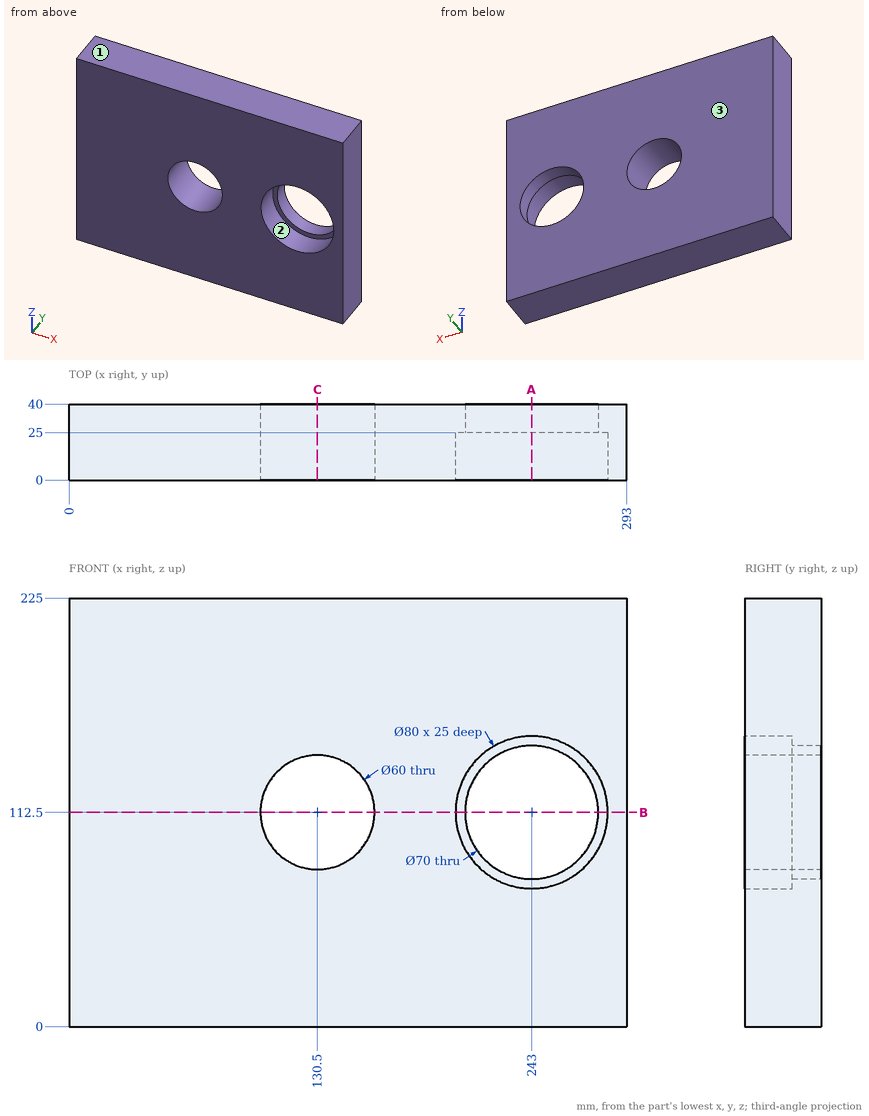
Input: dimensioned drawing with shaded views. Units: mm. Origin: part minimum x, y, z. Give positions to 0.01 mm unless a question says otherwise; leave off trailing zeros. Loops run counter-clockwise (first coordinate to the right, second up) from the corner with the lowest first, then second, coordinate; pieces in that order, holes last. Notation, with made-up numbers: (-7.75, -21) -> (22.25, -21) arc R21 cw to (22.25, 6) -> close; hole circle Ø11 at (-38.5, 42). An arc over 180 degrees is marked (long way). Use a Markdown table: item, result.
Q1. Section query A-A, the plane x = 243. Return the cut outline in (y, z).
Entries:
| item | result |
|---|---|
| outline | (0, 0) -> (40, 0) -> (40, 77.5) -> (25, 77.5) -> (25, 72.5) -> (0, 72.5) -> close; (0, 152.5) -> (25, 152.5) -> (25, 147.5) -> (40, 147.5) -> (40, 225) -> (0, 225) -> close |
Q2. Section query C-C, the plane x = 130.5. Return the cut outline in (y, z).
Entries:
| item | result |
|---|---|
| outline | (0, 0) -> (40, 0) -> (40, 82.5) -> (0, 82.5) -> close; (0, 142.5) -> (40, 142.5) -> (40, 225) -> (0, 225) -> close |
Q3. Pull-direction query (Z, two-part tool) for the marked faces 1, 2 and 3; classes: pulls with the +Z half, pulls with the -Z half, needs draft (parallel to the pull), parting line crosses it, or undercut.
Entries:
| item | result |
|---|---|
| face 1 | pulls with the +Z half |
| face 2 | undercut |
| face 3 | needs draft |
Q4. First-contact query: P1, Ø5, axis at y = 16, z = 58, coming from the -X side; P2, Ø10, axis at x = 239.5, z = 78, coming from the -Y side. Flat tips, straight axial feed; report the tip coordinate or a pass-through.
Entries:
| item | result |
|---|---|
| P1 | stops at x = 0 |
| P2 | stops at y = 25 |
Q5. Section query B-B, the plane z = 112.5. Return the cut outline in (x, y).
Entries:
| item | result |
|---|---|
| outline | (0, 0) -> (100.5, 0) -> (100.5, 40) -> (0, 40) -> close; (160.5, 0) -> (203, 0) -> (203, 25) -> (208, 25) -> (208, 40) -> (160.5, 40) -> close; (278, 25) -> (283, 25) -> (283, 0) -> (293, 0) -> (293, 40) -> (278, 40) -> close |
Q6. Ray query, probe 1 along X at (y, z) = (37, 112.5); probe 2 along X at (y, z) = (18, 112.5); probe 3 along Z at (x, y) = (132.5, 14.5). Return the intervals inside material, ascending. Write a range as from..to.
Entries:
| item | result |
|---|---|
| probe 1 | x = 0..100.5, 160.5..208, 278..293 |
| probe 2 | x = 0..100.5, 160.5..203, 283..293 |
| probe 3 | z = 0..82.57, 142.43..225 |
